Source: CAD feature listing. Evaluate the final solid. Frame: model axes, mm. A direction names the side the tool comes from. Round coordinates to 2 decimals unless told otherwise and drop trailing zeros. Loops run counter-clockwise (first coordinate to the right, second up) from the corner with the lowest first, then second, coordinate; pieces in that order, holes last. Notation, with made-up numbers: M 82.25,77.5 L 114.25,77.5 A23 ccw 114.25,111.5 Z; hole C 84,87 d1. An arc over 180 degrees is marked long. One line per item, written item: value.
from build123d import *

# Parameters (mm, degrees)
SKETCH_1_R        = 11
SKETCH_1_R_2      = 8
EXTRUDE_1_DEPTH   = 12.705
EXTRUDE_START     = -3
SKETCH_2_R        = 25
SKETCH_2_R_2      = 8
SKETCH_2_R_3      = 3
EXTRUDE_1_2_DEPTH = 3


with BuildPart() as part:
    # 草图1 → Extrude 1 (new, symmetric)
    with BuildSketch(Plane.XY):
        Circle(SKETCH_1_R)
        Circle(SKETCH_1_R_2, mode=Mode.SUBTRACT)
    extrude(amount=EXTRUDE_1_DEPTH, both=True)

    # 草图2 → Extrude 1 2 (add)
    with BuildSketch(Plane.XY.offset(12.705).offset(EXTRUDE_START)):
        Circle(SKETCH_2_R)
        Circle(SKETCH_2_R_2, mode=Mode.SUBTRACT)
        with Locations((0, 20)):
            Circle(SKETCH_2_R_3, mode=Mode.SUBTRACT)
        with Locations((20, 0)):
            Circle(SKETCH_2_R_3, mode=Mode.SUBTRACT)
        with Locations((0, -20)):
            Circle(SKETCH_2_R_3, mode=Mode.SUBTRACT)
        with Locations((-20, 0)):
            Circle(SKETCH_2_R_3, mode=Mode.SUBTRACT)
    extrude_1_2 = extrude(amount=EXTRUDE_1_2_DEPTH)

    # 镜向1: Extrude 1 2 across plane
    add(extrude_1_2.mirror(Plane.XY))


solid = part.part
1. Section query A-A (x = 20). Return the cut outline in (y, z) (3 decimals), and give its area (3 significant figures).
Report:
outline: M -15,-12.705 L -3,-12.705 L -3,-9.705 L -15,-9.705 Z; M -15,9.705 L -3,9.705 L -3,12.705 L -15,12.705 Z; M 3,-12.705 L 15,-12.705 L 15,-9.705 L 3,-9.705 Z; M 3,9.705 L 15,9.705 L 15,12.705 L 3,12.705 Z
area: 144 mm2
2. Section query B-B (y = 0). Count the separate pieces of the cut face and the enclosed holes in it, and give its area (3 significant figures).
Report:
separate pieces: 6
enclosed holes: 0
area: 248 mm2
3. Pin query (flat end, axial travel): pin 1 (3.5 mm diameter, centred on x = 0, y = 20, fed in from -Z); pin 2 (12 mm diameter, centred on x = -7, z = 2, fed in from -Y); pin 3 (1 mm diameter, centred on y = -2, z = 9.5, fed in from -X); pin 4 (4 mm diameter, centred on x = 10.5, z = -3, fed in from -Y). Return the tip coordinate at first contact, or that it passes through.
Report:
pin 1: passes through
pin 2: stops at y = -10.95
pin 3: stops at x = -24.95
pin 4: stops at y = -6.98
4. Reachability of faces 1 (the face through (5, -11, -9.705)), 2 (the face through (-0.65, 17.07, 11.18)) from +Z, -Z, +X, -X, +Y, -Y: full face, straight path, thin tool, end or side. Return the list, or none.
Report:
face 1: none
face 2: +Z, -Z
5. Pull-direction query (Y, two-part tool) for faces 3 (the face through (-1.73, -7.81, -0.18)), 4 (the face through (5, -11, 9.705)), 5 (the face through (23.846, 7.509, 11.184)); classes: released by +Y, released by -Y, zero draft, split by the parting line, or undercut.
Report:
face 3: undercut
face 4: zero draft
face 5: split by the parting line
6. Ray query, line 1 (Y direction, x = 0, z = 10.8); line 2 (Z direction, x = 18, y = -6.5) (3 decimals); line 3 (X direction, y = 0.5, z = -10.75) (3 decimals). Return the intervals inside material, ascending. Write a range as [from, to].
Report:
line 1: y = [-25, -23], [-17, -8], [8, 17], [23, 25]
line 2: z = [-12.705, -9.705], [9.705, 12.705]
line 3: x = [-24.995, -22.958], [-17.042, -7.984], [7.984, 17.042], [22.958, 24.995]
